Geometry: see drawing. Coordinates: mm, zero at the bounding-box minimum. Coordinates: 2 decimals unless noted, no trailing zeros. Loops run counter-clockwise (first coordinate to the right, second up) from the corner with the lowest first, then second, coordinate; pieces in that order, holes last.
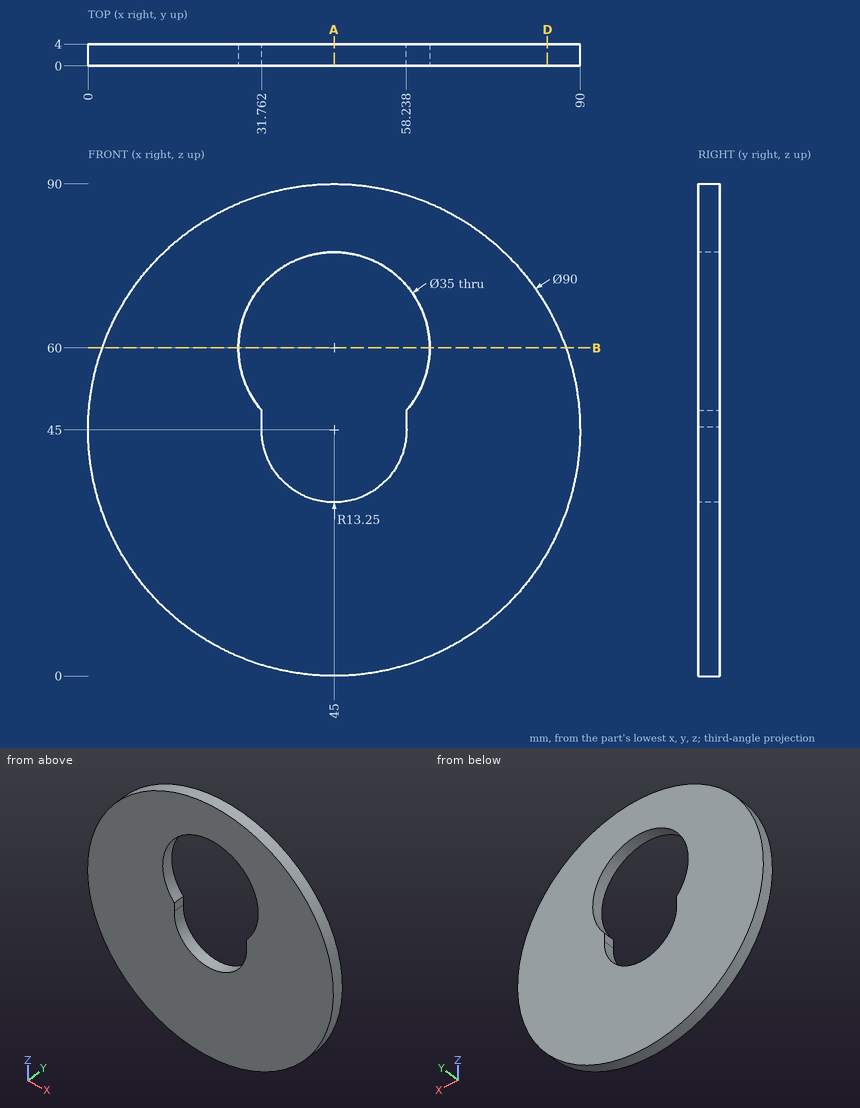
Item 1: Section query D-D (x = 84). Output: boundary loops of the cut face in (y, z), then the cut area to 3 significant figures.
Result:
outline: (0, 22.55) - (4, 22.55) - (4, 67.45) - (0, 67.45) - close
area: 180 mm2
Item 2: Line query: L1, parallel to X at y = 1.45, z = 73 (1 decimal); L2, parallel to Z at x = 40.5, y = 3.2 (1 decimal); L3, parallel to X at y = 3.5, z = 66.5. Output: solid intervals per line, ascending.
Result:
L1: x = 9.8 to 33.3, 56.7 to 80.2
L2: z = 0.2 to 32.5, 76.9 to 89.8
L3: x = 5.47 to 28.75, 61.25 to 84.53
Item 3: Section query A-A (x = 45). Output: boundary loops of the cut face in (y, z).
Result:
outline: (0, 0) - (4, 0) - (4, 31.75) - (0, 31.75) - close; (0, 77.5) - (4, 77.5) - (4, 90) - (0, 90) - close
Item 4: Contact query for flat-ended pins moving along their axis: P1, Ø2, axis at y = 0.5, z = 77.5, coming from the -X side (1 decimal); P2, Ø1.5, axis at y = 2, z = 47, coming from the +X side. Output: stop coordinate, or through.
Result:
P1: stops at x = 12.9
P2: stops at x = 89.98
Item 5: Section query B-B (z = 60). Output: boundary loops of the cut face in (x, y).
Result:
outline: (2.57, 0) - (27.5, 0) - (27.5, 4) - (2.57, 4) - close; (62.5, 0) - (87.43, 0) - (87.43, 4) - (62.5, 4) - close
